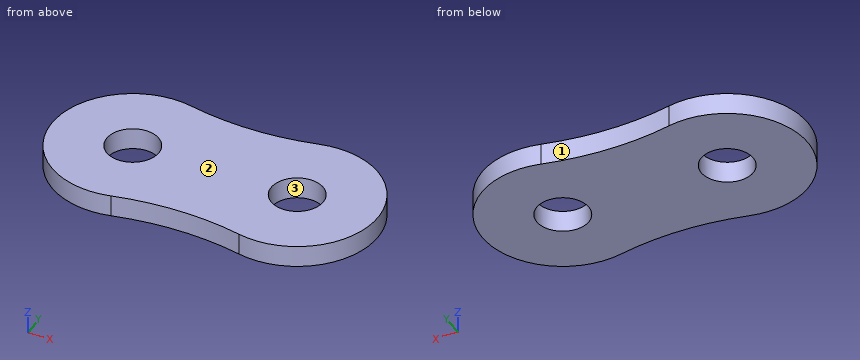
from build123d import *

# Parameters (mm, degrees)
EXTRUDE_1_DEPTH     = 1.665
SKETCH_3_R          = 1.99
CUT_EXTRUDE_1_DEPTH = 15.050077402


with BuildPart() as part:
    # 草图2 → 拉伸1 (new body)
    with BuildSketch(Plane.XY):
        with BuildLine():
            ThreePointArc((-4.944493019, 6.002647343), (-12.515, 0), (-4.944493019, -6.002647343))
            ThreePointArc((-4.944493019, -6.002647343), (0, -5.4315), (4.944493019, -6.002647343))
            ThreePointArc((4.944493019, -6.002647343), (12.515, 0), (4.944493019, 6.002647343))
            ThreePointArc((4.944493019, 6.002647343), (0, 5.4315), (-4.944493019, 6.002647343))
        make_face()
    extrude(amount=EXTRUDE_1_DEPTH)

    # 草图3 → 切除-拉伸1 (cut, through all)
    with BuildSketch(Plane.XY.offset(1.665)):
        with Locations((-6.35, 0)):
            Circle(SKETCH_3_R)
        with Locations((6.35, 0)):
            Circle(SKETCH_3_R)
    extrude(amount=-CUT_EXTRUDE_1_DEPTH, mode=Mode.SUBTRACT)


solid = part.part
Read the model definition and answer for the solid it produces. Units are mm, in the model's axes. Face numbers are marked on the shaded views. Coordinates: 2 decimals unless noted, no trailing zeros. Order: outer loops, then holes, each group sorted by start corner. A loop starts at its lowest first (then second) coordinate and runs counter-clockwise, first axis right, second up. Notation, with made-up numbers: (-28.5, 84.25) - (-14.5, 84.25) arc R31 ccw to (-14.5, 122.25) - close; hole circle Ø3 at (77.5, 58). An arc over 180 degrees is marked (long way). Use one line per item in the form item = value.
(1) Section D-D, the plane x = 6.25 is taken. Give the vertices of the cut face in (y, z) (3 decimals).
Computed values:
outline = (-6.164, 0) - (-1.987, 0) - (-1.987, 1.665) - (-6.164, 1.665) - close; (1.987, 0) - (6.164, 0) - (6.164, 1.665) - (1.987, 1.665) - close
(2) Section A-A, the plane y = 0 is taken. Give the vertices of the cut face in (x, z) (3 decimals).
Computed values:
outline = (-12.515, 0) - (-8.34, 0) - (-8.34, 1.665) - (-12.515, 1.665) - close; (-4.36, 0) - (4.36, 0) - (4.36, 1.665) - (-4.36, 1.665) - close; (8.34, 0) - (12.515, 0) - (12.515, 1.665) - (8.34, 1.665) - close
(3) For a pull along X with two mould halves and no side action, classify the marked faces 1, 2 and 3 as pulls with the +X half, pulls with the -X half, needs draft (parallel to the pull), parting line crosses it, or undercut.
Computed values:
face_1 = undercut
face_2 = needs draft
face_3 = undercut
(4) Straight lines are drawn through the part: L1, parallel to Y at x = 6.35, z = 1 (3 decimals); L2, parallel to X at y = 1.5, z = 1.2; L3, parallel to X at y = -1, z = 1.45. For each, find the intervals that lie inside material, in ascending order.
Computed values:
L1 = -6.165 to -1.99, 1.99 to 6.165
L2 = -12.33 to -7.66, -5.04 to 5.04, 7.66 to 12.33
L3 = -12.43 to -8.07, -4.63 to 4.63, 8.07 to 12.43
(5) Section C-C, the plane z = 0.35 is taken. Give the number of separate pieces and of enclosed holes in the cut face, then the cut area to 3 significant figures.
Computed values:
separate_pieces = 1
enclosed_holes = 2
area = 240 mm²
(6) Section B-B, the plane x = -6.35 is taken. Give the vertices of the cut face in (y, z) (3 decimals).
Computed values:
outline = (-6.165, 0) - (-1.99, 0) - (-1.99, 1.665) - (-6.165, 1.665) - close; (1.99, 0) - (6.165, 0) - (6.165, 1.665) - (1.99, 1.665) - close
